Design review of the part shown in the three views and the two pictorial views. Dimensions are in mm from the part's minimum x, y and z. Round coordinates to 2 decimals unless told otherwise and drop trailing zeros. Write each loop counter-clockwise with the first axis right and the second up, starting at its lowest first coordinate (ties: lowest second). Pieces come first, ordered by that corner, then holes. Notation, with made-up numbers: (-14.75, 80) -> (-6.75, 80) arc R26 ccw to (-6.75, 98) -> close; hole circle Ø9 at (54, 10.25). An arc over 180 degrees is marked (long way). Return JSON: item names as keys, results as strings. Group by question number.
1. Take a section at B-B, the plane z = 0.6. Write out the cut boundary in (x, y) (1 decimal).
2. For line 1 along Y through (x, z) = (5.25, 2.3); line 2 along Y through (x, z) = (6.25, 1.95); line 3 along X through (y, z) = (4, 3.1) (1 decimal), list the stretches that pass through material, from the lowest coordinate up. Write a range as from..to.
3. Clearance check with flat-ended pins moving along their axes: P1, Ø1.5, axis at x = 3.5, z = 2, coming from the +Y side; P2, Ø1, axis at y = 7, z = 3.5, coming from the +X side (1 decimal). State where each tip first meets the part, or that it passes through.
4. Mouldability with a two-part tool opening along X and no side actions: class the marked faces 1, 2, 3 and 4 as pulls with the +X half, pulls with the -X half, needs draft (parallel to the pull), parting line crosses it, or undercut.
5. Take a section at A-A, the plane z = 1.4. Write out the cut boundary in (x, y) (1 decimal), then the cut area to 3 significant figures.
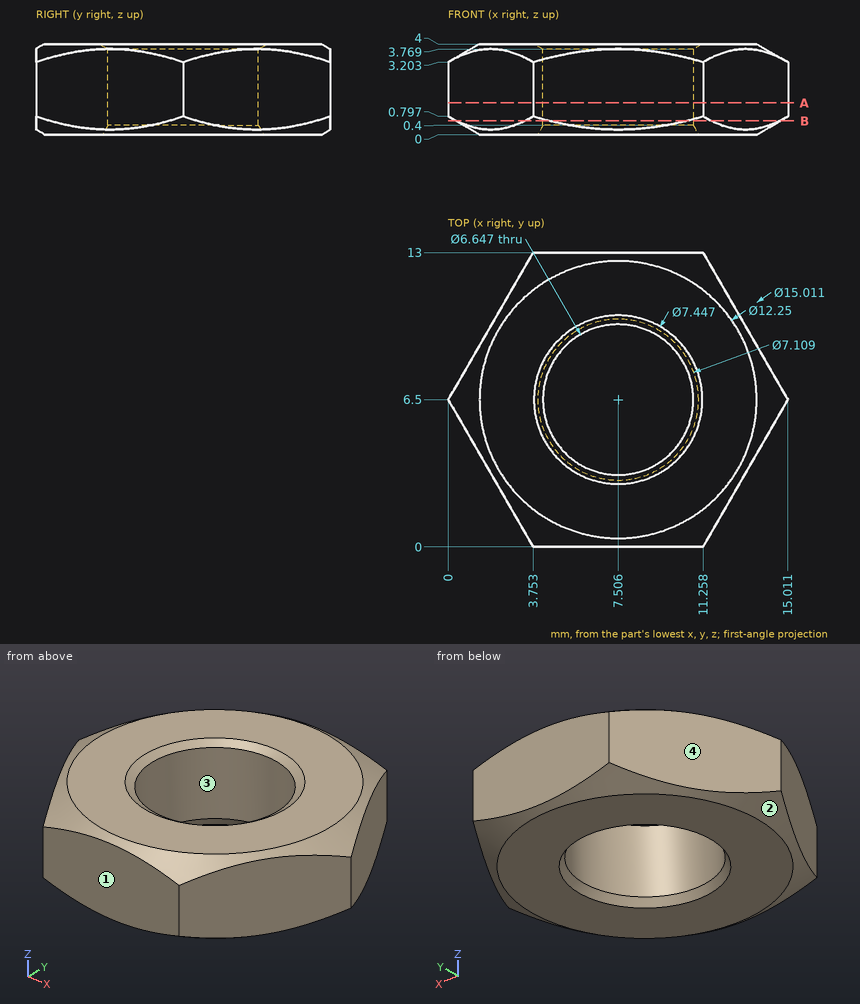
Output:
{
 "1": {"outline": "(0.4, 5.9) -> (3.4, 0.6) arc R7.2 ccw to (4.5, 0) -> (10.5, 0) arc R7.2 ccw to (11.6, 0.6) -> (14.6, 5.9) arc R7.2 ccw to (14.6, 7.1) -> (11.6, 12.4) arc R7.2 ccw to (10.5, 13) -> (4.5, 13) arc R7.2 ccw to (3.4, 12.4) -> (0.4, 7.1) arc R7.2 ccw to start; hole circle Ø6.6 at (7.5, 6.5)"},
 "2": {"line 1": "y = 0..4.06, 8.94..13", "line 2": "y = 0..3.42, 9.58..13", "line 3": "x = 1.4..5.3, 9.7..13.6"},
 "3": {"P1": "stops at y = 13", "P2": "stops at x = 15"},
 "4": {"face 1": "needs draft", "face 2": "parting line crosses it", "face 3": "undercut", "face 4": "pulls with the -X half"},
 "5": {"outline": "(0, 6.5) -> (3.8, 0) -> (11.3, 0) -> (15, 6.5) -> (11.3, 13) -> (3.8, 13) -> close; hole circle Ø6.6 at (7.5, 6.5)", "area": "112 mm^2"}
}
